Source: CAD feature listing. Evaluate the final solid. Frame: model axes, mm. A direction names the side the tool comes from. Give positions to 0.01 mm unless a question says otherwise; leave off trailing zeros. Loops run counter-clockwise (first coordinate to the right, second up) from the corner with the lowest first, then second, coordinate; pieces in that order, holes last. Notation, with made-up numbers: (-15, 54) -> (41, 54) arc R20 cw to (41, 90) -> close; hole circle Ø2 at (-13, 78.5). An arc over 180 degrees is marked (long way). Put each result on its own line as item: value.
```python
from build123d import *

# Parameters (mm, degrees)
SKETCH1_W           = 30
SKETCH1_H           = 30
BOSS_EXTRUDE1_DEPTH = 800
SKETCH2_W           = 24
SKETCH2_H           = 24
CUT_EXTRUDE1_DEPTH  = 800
CUT_EXTRUDE2_DEPTH  = 802.704175948
SKETCH4_R           = 3
CUT_EXTRUDE3_DEPTH  = 754.969037173


with BuildPart() as part:
    # Sketch1 → Boss-Extrude1 (new body)
    with BuildSketch(Plane.XY):
        with Locations((-27.773656986, 31.621806058)):
            Rectangle(SKETCH1_W, SKETCH1_H)
    extrude(amount=BOSS_EXTRUDE1_DEPTH)

    # Sketch2 → Cut-Extrude1 (cut)
    with BuildSketch(Plane.XY.offset(800)):
        with Locations((-27.773656986, 31.621806058)):
            Rectangle(SKETCH2_W, SKETCH2_H)
    extrude(amount=-CUT_EXTRUDE1_DEPTH, mode=Mode.SUBTRACT)

    # Sketch3 → Cut-Extrude2 (cut, through all)
    with BuildSketch(Plane(origin=(0, 16.621806058, 0), x_dir=(-1, 0, 0), z_dir=(0, -1, 0))):
        Polygon((12.773656986, -721.664630148), (42.773656986, -751.664630148), (42.773656986, -800), (12.773656986, -800), align=None)
        Polygon((12.773656986, -155.979205198), (42.773656986, -125.979205198), (42.773656986, 0), (12.773656986, 0), align=None)
    extrude(amount=-CUT_EXTRUDE2_DEPTH, mode=Mode.SUBTRACT)

    # Sketch4 → Cut-Extrude3 (cut, through all)
    with BuildSketch(Plane.ZY.offset(48.773656986)):
        with Locations(Location((225.979205198, 31.621806058, 0), (0, 0, 270))):
            Circle(SKETCH4_R)
        with Locations((225.979205198, 841.621806058)):
            Circle(SKETCH4_R)
        with Locations((651.664630148, 841.621806058)):
            Circle(SKETCH4_R)
        with Locations(Location((651.664630148, 31.621806058, 0), (0, 0, 269.999999999))):
            Circle(SKETCH4_R)
    extrude(amount=-CUT_EXTRUDE3_DEPTH, mode=Mode.SUBTRACT)


solid = part.part
```
(1) Draft query along X for faces 3 (the flat face through (-12.774, 31, 435)), 4 (the flat face through (-28, 46.622, 434)), 5 (the flat face through (-28, 43.622, 443)). Return one class per face: released by +X, released by -X, zero draft, split by the parting line, or undercut.
Calculated:
face 3: released by +X
face 4: zero draft
face 5: undercut
(2) Section A-A on z = 295. Return loops of the section in (x, y).
Calculated:
outline: (-42.77, 16.62) -> (-12.77, 16.62) -> (-12.77, 46.62) -> (-42.77, 46.62) -> close; hole (-39.77, 19.62) -> (-15.77, 19.62) -> (-15.77, 43.62) -> (-39.77, 43.62) -> close
(3) Reachability of faces 1 (the flat face through (-28, 16.622, 434)), 2 (the flat face through (-15.774, 31, 443)) from +Z, -Z, +X, -X, +Y, -Y: full face, straight path, thin tool, end or side. Return the list, or none.
Calculated:
face 1: +Z, -Z, +X, -X, -Y
face 2: +Z, -Z
(4) First-contact query: P1, Ø9.5, axis at y = 31.62, z = 651.66, coming from the +X side. Flat tip, straight axial feed; report the tip coordinate or a pass-through.
Calculated:
P1: stops at x = -12.77
(5) Section B-B on x = -35. Return loops of the section in (y, z), then the cut area to 3 significant figures.
Calculated:
outline: (16.62, 133.75) -> (19.62, 133.75) -> (19.62, 743.89) -> (16.62, 743.89) -> close; (43.62, 133.75) -> (46.62, 133.75) -> (46.62, 743.89) -> (43.62, 743.89) -> close
area: 3,660 mm²
(6) Line query: probe 1 along Y at (x, z) = (-18, 375); probe 2 along X at (y, z) = (41, 537); probe 3 along Z at (x, y) = (-14, 33.5). Output: solid intervals per line, ascending. Write a range as from..to.
Calculated:
probe 1: y = 16.62..19.62, 43.62..46.62
probe 2: x = -42.77..-39.77, -15.77..-12.77
probe 3: z = 154.75..223.64, 228.32..649.33, 654..722.89
